from build123d import *

# Parameters (mm, degrees)
SKETCH_1_W          = 250
SKETCH_1_H          = 150
EXTRUDE_1_DEPTH     = 12
HOLE_WIZARD_M20_1_D = 17.5
HOLE_WIZARD_M8_1_D  = 6.8
FILLET_1_R          = 10


with BuildPart() as part:
    # 草图1 → 凸台-拉伸1 (new body)
    with BuildSketch(Plane(origin=(0, 0, 0), x_dir=(1, 0, 0), z_dir=(0, 1, 0))):
        Rectangle(SKETCH_1_W, SKETCH_1_H)
    extrude(amount=EXTRUDE_1_DEPTH)

    # M20 螺纹孔1 (through all)
    with Locations(Plane(origin=(0, 0, 0), x_dir=(-1, 0, 0), z_dir=(0, -1, 0))):
        with Locations((100, -50)):
            Hole(HOLE_WIZARD_M20_1_D / 2)

    # M8 螺纹孔1 (through all)
    with Locations(Plane(origin=(0, 12, 0), x_dir=(1, 0, 0), z_dir=(0, 1, 0))):
        with Locations((25.5, 54.5), (104.5, 54.5), (25.5, -24.5), (104.5, -24.5)):
            Hole(HOLE_WIZARD_M8_1_D / 2)

    # 圆角1
    fillet_1_edges = [part.edges().sort_by_distance(p)[0] for p in [
        (125, 6, 75),
        (-125, 6, 75),
        (-125, 6, -75),
        (125, 6, -75),
    ]]
    fillet(fillet_1_edges, radius=FILLET_1_R)


solid = part.part
Verification items for the finished model (mm, model axes). Give positions to 0.01 mm unless a question says otherwise; leave off trailing zeros. Write each loop counter-clockwise with the first axis right and the second up, starting at its lowest first coordinate (ties: lowest second). Pieces come first, ordered by that corner, then holes. Notation, with made-up numbers: M 36,31 L 65,31 A27 cw 65,48 Z; hole C -23.75,61.5 d7. An arc over 180 degrees is marked long. Use CSV: the item, a comma, the result in double quotes.
1) Cross-section at A-A (z = 24.5). Enter the section's corners in (x, y), plus the area to 3 significant figures.
Final values:
outline,"M -125,0 L 22.1,0 L 22.1,12 L -125,12 Z; M 28.9,0 L 101.1,0 L 101.1,12 L 28.9,12 Z; M 107.9,0 L 125,0 L 125,12 L 107.9,12 Z"
area,"2,840 mm²"
2) Cross-section at C-C (x = -100). Enter the section's corners in (y, z).
Final values:
outline,"M 0,-75 L 12,-75 L 12,41.25 L 0,41.25 Z; M 0,58.75 L 12,58.75 L 12,75 L 0,75 Z"
3) Release check for a two-part mould opening along X. For faces 1 (the face through (107.9, 5.9, -54.6)), 2 (the face through (-106.944, 6.084, 55.324)), 3 (the face through (-2, 6, 75)), 4 (the face through (121.99, 6.08, -72.15)) record: released by +X, released by -X, zero draft, split by the parting line, or undercut.
Final values:
face 1,"undercut"
face 2,"undercut"
face 3,"zero draft"
face 4,"released by +X"
4) Material ranges on line 1 along X through (y, z) = (9.25, 24.5); line 2 along Z through (x, y) = (25.5, 7); line 3 along X through (y, z) = (7, 50), recorded low to high.
Final values:
line 1,"-125 to 22.1, 28.9 to 101.1, 107.9 to 125"
line 2,"-75 to -57.9, -51.1 to 21.1, 27.9 to 75"
line 3,"-125 to -108.75, -91.25 to 125"
5) Cross-section at B-B (x = 104.5). Enter the section's corners in (y, z).
Final values:
outline,"M 0,-75 L 12,-75 L 12,-57.9 L 0,-57.9 Z; M 0,-51.1 L 12,-51.1 L 12,21.1 L 0,21.1 Z; M 0,27.9 L 12,27.9 L 12,75 L 0,75 Z"
